from build123d import *

# Parameters (mm, degrees)
SKETCH1_W                                            = 150
SKETCH1_H                                            = 270
BOSS_EXTRUDE1_DEPTH                                  = 6
SKETCH2_R                                            = 10
CUT_EXTRUDE1_DEPTH                                   = 2
M10_CLEARANCE_HOLE1_D                                = 11
SKETCH5_R                                            = 7.5
CUT_EXTRUDE2_DEPTH                                   = 2
HOLE_SIZE_PER_SOCKET_HEAD_CAP_SCREW_TYPE_D           = 6.6
HOLE_SIZE_PER_SOCKET_HEAD_CAP_SCREW_TYPE_CBORE_D     = 11
HOLE_SIZE_PER_SOCKET_HEAD_CAP_SCREW_TYPE_CBORE_DEPTH = 6.8
M8_TAPPED_HOLE2_D                                    = 6.8
CHAMFER1_SIZE                                        = 0.5
M8_CLEARANCE_HOLE1_D                                 = 9


with BuildPart() as part:
    # Sketch1 → Boss-Extrude1 (new, symmetric)
    with BuildSketch(Plane(origin=(0, 0, 0), x_dir=(1, 0, 0), z_dir=(0, 1, 0))):
        Rectangle(SKETCH1_W, SKETCH1_H)
    extrude(amount=BOSS_EXTRUDE1_DEPTH, both=True)

    # Sketch2 → Cut-Extrude1 (cut)
    with BuildSketch(Plane.XZ.offset(6)):
        with Locations(Location((-53, 110, 0), (0, 0, 270))):
            Circle(SKETCH2_R)
        with Locations(Location((53, 110, 0), (0, 0, 90))):
            Circle(SKETCH2_R)
        with Locations(Location((53, -110, 0), (0, 0, 270))):
            Circle(SKETCH2_R)
        with Locations(Location((-53, -110, 0), (0, 0, 90))):
            Circle(SKETCH2_R)
    extrude(amount=-CUT_EXTRUDE1_DEPTH, mode=Mode.SUBTRACT)

    # M10 Clearance Hole1 (through all)
    with Locations(Plane(origin=(0, 6, 0), x_dir=(1, 0, 0), z_dir=(0, 1, 0))):
        with Locations((-53, 110), (53, 110), (-53, -110), (53, -110)):
            Hole(M10_CLEARANCE_HOLE1_D / 2)

    # Sketch5 → Cut-Extrude2 (cut)
    with BuildSketch(Plane(origin=(0, 6, 0), x_dir=(1, 0, 0), z_dir=(0, 1, 0))):
        with Locations(Location((-20, 125, 0), (0, 0, 270))):
            Circle(SKETCH5_R)
        with Locations(Location((20, 125, 0), (0, 0, 90))):
            Circle(SKETCH5_R)
        with Locations(Location((20, -125, 0), (0, 0, 270))):
            Circle(SKETCH5_R)
        with Locations(Location((-20, -125, 0), (0, 0, 90))):
            Circle(SKETCH5_R)
    extrude(amount=-CUT_EXTRUDE2_DEPTH, mode=Mode.SUBTRACT)

    # Hole size per socket head cap screw type 1 (through all)
    with Locations(Plane(origin=(0, -6, 0), x_dir=(-1, 0, 0), z_dir=(0, -1, 0))):
        with Locations((20, -125), (-20, -125), (20, 125), (-20, 125)):
            CounterBoreHole(HOLE_SIZE_PER_SOCKET_HEAD_CAP_SCREW_TYPE_D / 2, HOLE_SIZE_PER_SOCKET_HEAD_CAP_SCREW_TYPE_CBORE_D / 2, HOLE_SIZE_PER_SOCKET_HEAD_CAP_SCREW_TYPE_CBORE_DEPTH)

    # M8 Tapped Hole2 (through all)
    with Locations(Plane(origin=(0, -6, 0), x_dir=(-1, 0, 0), z_dir=(0, -1, 0))):
        with Locations((21, 19), (21, -19), (-21, -19), (-21, 19)):
            Hole(M8_TAPPED_HOLE2_D / 2)

    # Chamfer1
    chamfer1_edges = [part.edges().sort_by_distance(p)[0] for p in [
        (75, 0, 135),
        (-75, 0, 135),
        (-75, 0, -135),
        (75, 0, -135),
    ]]
    chamfer(chamfer1_edges, length=CHAMFER1_SIZE)

    # M8 Clearance Hole1 (through all)
    with Locations(Plane(origin=(0, 6, 0), x_dir=(1, 0, 0), z_dir=(0, 1, 0))):
        with Locations((27.5, 46.7), (-27.5, 46.7), (27.5, -63.3), (-27.5, -63.3)):
            Hole(M8_CLEARANCE_HOLE1_D / 2)


solid = part.part
The model under review builds one solid part; all positions refer to its coordinate system, in mm. A direction names the side the tool comes from. Round coordinates to 2 decimals unless told otherwise and drop trailing zeros. Write each loop counter-clockwise with the first axis right and the second up, starting at its lowest first coordinate (ties: lowest second). Pieces come first, ordered by that corner, then holes. Notation, with made-up numbers: (-0.75, 35.5) - (43.25, 35.5) arc R8 cw to (43.25, 46.5) - close; hole circle Ø8 at (73.25, 78). An arc over 180 degrees is marked (long way). One line per item, written item: value. Start each with the question number.
1. The part is to be moulded in two halves that separate along X. For faces 4 (the face through (22, 4, -128)), 5 (the face through (-22.253, 5.014, 117.846)), 6 (the face through (-1, 0, 135)), say which applies: released by +X, released by -X, zero draft, split by the parting line, or undercut.
2. Consider section A-A on z = 125. Write out the cut boundary in (x, y), and give its area (3 significant figures).
3. To check wall thickness, follow L1, parallel to X at y = 5, z = 125; L2, parallel to Z at x = -53, y = 1; L3, parallel to X at y = 3.1, z = 125. State the ranges of each line that lie inside material, in increasing order. Write a range as from..to.
4. Consider section D-D on x = 50.5. Write out the cut boundary in (y, z).
5. Consider section C-C on z = -46.7. Write out the cut boundary in (x, y), and give its area (3 significant figures).
6. Clearance check with flat-ended pins moving along their axes: P1, Ø10, axis at x = 53, z = -110, coming from the +Y side; P2, Ø10, axis at x = 20, z = -125, coming from the -Y side; P3, Ø5.5, axis at x = -18.5, z = 122.5, coming from the -Y side; P4, Ø7.5, axis at x = 19.5, z = 122, coming from the +Y side. State where each tip first meets the part, or that it passes through.
7. Consider section B-B on x = -53. Write out the cut boundary in (y, z).
8. Machinability: for faces 1 (the face through (-47, -5, -118)), 2 (the face through (-20.72, 2.42, -121.78)), 3 (the face through (22.253, 5.014, 132.154)), which of the approach directions +Z, -Z, +X, -X, +Y, -Y give a long, thin tool a straight path to every point of the face, cutting with its end or side? Answer none if there is none.
Checks:
1. face 4: undercut
1. face 5: undercut
1. face 6: zero draft
2. outline: (-75, -6) - (-25.5, -6) - (-25.5, 0.8) - (-23.3, 0.8) - (-23.3, 4) - (-27.5, 4) - (-27.5, 6) - (-75, 6) - close; (-16.7, 0.8) - (-14.5, 0.8) - (-14.5, -6) - (14.5, -6) - (14.5, 0.8) - (16.7, 0.8) - (16.7, 4) - (12.5, 4) - (12.5, 6) - (-12.5, 6) - (-12.5, 4) - (-16.7, 4) - close; (23.3, 0.8) - (25.5, 0.8) - (25.5, -6) - (75, -6) - (75, 6) - (27.5, 6) - (27.5, 4) - (23.3, 4) - close
2. area: 1,550 mm^2
3. L1: x = -75..-27.5, -12.5..12.5, 27.5..75
3. L2: z = -135..-115.5, -104.5..104.5, 115.5..135
3. L3: x = -75..-23.3, -16.7..16.7, 23.3..75
4. outline: (-6, -135) - (6, -135) - (6, -114.9) - (-4, -114.9) - (-4, -119.68) - (-6, -119.68) - close; (-6, -100.32) - (-4, -100.32) - (-4, -105.1) - (6, -105.1) - (6, 105.1) - (-4, 105.1) - (-4, 100.32) - (-6, 100.32) - close; (-6, 119.68) - (-4, 119.68) - (-4, 114.9) - (6, 114.9) - (6, 135) - (-6, 135) - close
5. outline: (-75, -6) - (-32, -6) - (-32, 6) - (-75, 6) - close; (-23, -6) - (23, -6) - (23, 6) - (-23, 6) - close; (32, -6) - (75, -6) - (75, 6) - (32, 6) - close
5. area: 1,580 mm^2
6. P1: passes through
6. P2: stops at y = 0.8
6. P3: stops at y = -6
6. P4: stops at y = 4
7. outline: (-6, -135) - (6, -135) - (6, -115.5) - (-4, -115.5) - (-4, -120) - (-6, -120) - close; (-6, -100) - (-4, -100) - (-4, -104.5) - (6, -104.5) - (6, 104.5) - (-4, 104.5) - (-4, 100) - (-6, 100) - close; (-6, 120) - (-4, 120) - (-4, 115.5) - (6, 115.5) - (6, 135) - (-6, 135) - close
8. face 1: -Y
8. face 2: +Y, -Y
8. face 3: +Y
